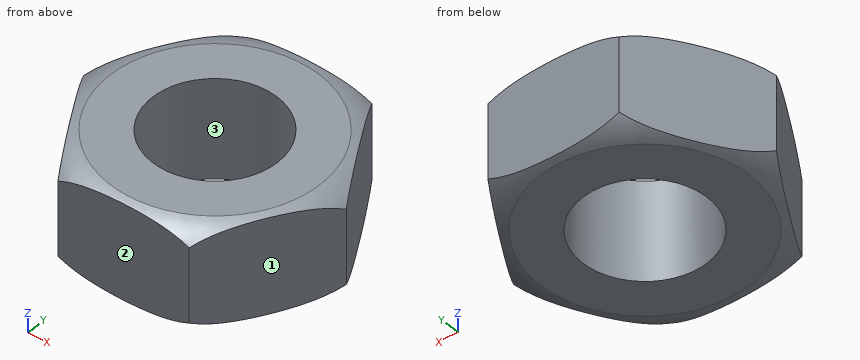
from build123d import *

# Parameters (mm, degrees)
SKETCH5_R           = 5
BOSS_EXTRUDE2_DEPTH = 8
SCALE_1_SCALE       = 1.875


with BuildPart() as part:
    # Sketch5 → Boss-Extrude2 (new body)
    with BuildSketch(Plane.XY):
        Polygon((10.392304845, 0), (5.196152423, 9), (-5.196152423, 9), (-10.392304845, 0), (-5.196152423, -9), (5.196152423, -9), align=None)
        Circle(SKETCH5_R, mode=Mode.SUBTRACT)
    extrude(amount=BOSS_EXTRUDE2_DEPTH)

    # Sketch6 → Cut-Revolve2 (revolve, cut)
    with BuildSketch(Plane(origin=(0, 0, 0), x_dir=(1, 0, 0), z_dir=(0, 1, 0))):
        with BuildLine():
            Line((-10.392304845, 0), (-10.392304845, -1))
            ThreePointArc((-10.392304845, -1), (-9.463602824, -0.357404043), (-8.392304845, 0))
            Line((-8.392304845, 0), (-10.392304845, 0))
        make_face()
        with BuildLine():
            Line((-10.392304845, -8), (-8.392304845, -8))
            ThreePointArc((-8.392304845, -8), (-9.463602824, -7.642595957), (-10.392304845, -7))
            Line((-10.392304845, -7), (-10.392304845, -8))
        make_face()
    revolve(axis=Axis((0, 0, 0), (0, 0, 1)), mode=Mode.SUBTRACT)


with BuildPart() as part_1:
    # Scale 1: scaled about (-5.25e-07, 1.59e-07, 3.999997472)
    add(part.part.scale(SCALE_1_SCALE).moved(Location((4.59e-07, -1.39e-07, -3.499997788))))


solid = part_1.part
Verification items for the finished model (mm, model axes). Face numbers are marked on the shaded views. Coordinates: 2 decimals unless noted, no trailing zeros. Write each loop counter-clockwise with the first axis right and the second up, starting at its lowest first coordinate (ties: lowest second). Pieces come first, ordered by that corner, then holes. Notation, with made-up numbers: M -9.5,79.25 L 6.5,79.25 A22 ccw 6.5,112.25 Z; hole C 79,3.25 d9. An arc over 180 degrees is marked long. Use a Markdown table: item, result.
Q1. Go/stop test with flat-tipped pins: P1, Ø1, axis at y = -1.5, z = 9.5, coming from the +X side; P2, Ø1, axis at x = 12, z = 0, coming from the +Y side; P3, Ø5, axis at y = 8.5, z = 9.5, coming from the +X side. Record where each tip stops, or that it passes through.
Reply:
| item | result |
|---|---|
| P1 | stops at x = 18.91 |
| P2 | stops at y = 13.83 |
| P3 | stops at x = 16.02 |
Q2. Thickness scan on line 1 (Y direction, x = 0, z = 4.25) (3 decimals); line 2 (X direction, y = 0, z = 1.5) (3 decimals); line 3 (X direction, y = 4.5, z = 10). Record the ranges inside material, lowest first.
Reply:
| item | result |
|---|---|
| line 1 | y = -16.875 to -9.375, 9.375 to 16.875 |
| line 2 | x = -19.486 to -9.375, 9.375 to 19.486 |
| line 3 | x = -16.89 to -8.22, 8.22 to 16.89 |
Q3. Sectioned sample at A-A, the plane z = 3. Record the boundary of the cut face in (x, y) (3 decimals).
Reply:
| item | result |
|---|---|
| outline | M -19.486,0 L -9.743,-16.875 L 9.743,-16.875 L 19.486,0 L 9.743,16.875 L -9.743,16.875 Z; hole C 0,0 d18.75 |
Q4. Draft check along X on the marked faces 1, 2 and 3. Enter one of: +X half, -X half, draft (parallel to the pull), parting line (faces both ways), or undercut.
Reply:
| item | result |
|---|---|
| face 1 | +X half |
| face 2 | draft |
| face 3 | undercut |
